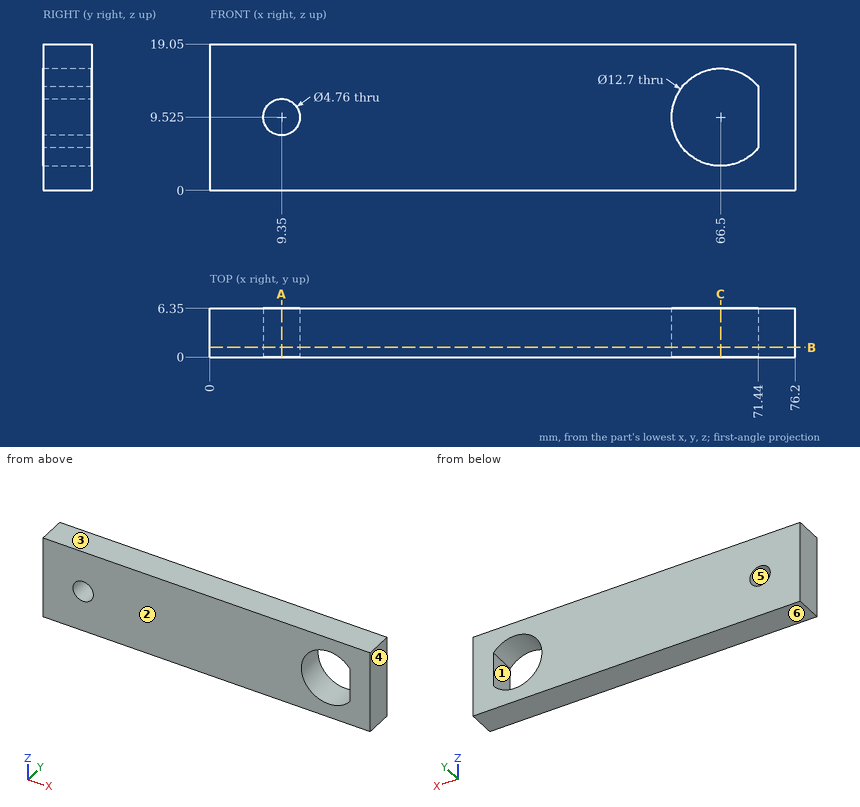
Verification items for this drawing (mm, ordinates from the low corner). A direction names the side the tool comes from. Coordinates: 2 decimals unless noted, no trailing zeros. Write each loop counter-clockwise with the first axis right and the second up, starting at its lowest first coordinate (ties: lowest second). Pieces come first, ordered by that corner, then holes. Notation, with made-up numbers: M 33.25,-6 L 49.25,-6 A16 cw 49.25,12 Z; hole C 57.5,2.5 d6. An arc over 180 degrees is marked long. Answer as a JSON object with one key per item and string values. Group by question number.
(1) Cross-section at B-B, the plane y = 1.25. Record the cut outline in (x, z) (3 decimals).
(2) Gauge pin test, flat end, axial feed: pin 1 (10 mm diameter, centred on x = 46.5, z = 10, fed in from -Y). Record the tip position at first contact, or that the pin passes through.
(3) Tool access check on the marked faces 1 and 2. Record the directions out of +Z, -Z, +X, -X, +Y, -Y that give a thin tool (end or side, any length) a straight path to the whole face; none if there is none.
(4) Release check for a two-part mould opening along Z. For the marked faces 3, 4, 5 and 6 record: +Z half, -Z half, draft (parallel to the pull), parting line (faces both ways), or undercut.
(5) Material ranges on line 1 (Z direction, x = 66.5, y = 2) (3 decimals); line 2 (X direction, y = 2.75, z = 7.5); line 3 (X direction, y = 6, z = 11), recorded low to high.
(6) Cross-section at C-C, the plane x = 66.5. Record the cut outline in (y, z) (3 decimals).
(7) Cross-section at A-A, the plane x = 9.35. Record the cut outline in (y, z) (3 decimals).
Reply:
{
 "1": {"outline": "M 0,0 L 76.2,0 L 76.2,19.05 L 0,19.05 Z; hole C 9.35,9.525 d4.76; hole M 71.44,5.535 L 71.44,13.515 A6.35 ccw long Z"},
 "2": {"pin 1": "y = 0"},
 "3": {"face 1": "+Y, -Y", "face 2": "+Z, -Z, +X, -X, -Y"},
 "4": {"face 3": "+Z half", "face 4": "draft", "face 5": "undercut", "face 6": "-Z half"},
 "5": {"line 1": "0 to 3.175, 15.875 to 19.05", "line 2": "0 to 8.1, 10.6 to 60.48, 71.44 to 76.2", "line 3": "0 to 7.48, 11.22 to 60.32, 71.44 to 76.2"},
 "6": {"outline": "M 0,0 L 6.35,0 L 6.35,3.175 L 0,3.175 Z; M 0,15.875 L 6.35,15.875 L 6.35,19.05 L 0,19.05 Z"},
 "7": {"outline": "M 0,0 L 6.35,0 L 6.35,7.145 L 0,7.145 Z; M 0,11.905 L 6.35,11.905 L 6.35,19.05 L 0,19.05 Z"}
}
